from build123d import *

# Parameters (mm, degrees)
SKETCH1_W           = 800
SKETCH1_H           = 1200
BOSS_EXTRUDE1_DEPTH = 100
SKETCH2_W           = 40
SKETCH2_H           = 40
CUT_EXTRUDE1_DEPTH  = 1269.857754045
LPATTERN1_COUNT     = 5
LPATTERN1_PITCH     = 90
LPATTERN1_COL_COUNT = 5
LPATTERN1_COL_PITCH = 90


with BuildPart() as part:
    # Sketch1 → Boss-Extrude1 (new body)
    with BuildSketch(Plane.XY):
        Rectangle(SKETCH1_W, SKETCH1_H)
    extrude(amount=BOSS_EXTRUDE1_DEPTH)

    # Sketch2 → Cut-Extrude1 (cut, through all)
    with BuildSketch(Plane.XZ.offset(600)):
        with Locations((0, 100)):
            Rectangle(SKETCH2_W, SKETCH2_H)
    cut_extrude1 = extrude(amount=-CUT_EXTRUDE1_DEPTH, mode=Mode.SUBTRACT)

    # LPattern1: Cut-Extrude1 ×5
    with Locations(*[(i * LPATTERN1_PITCH, 0, 0) for i in range(1, LPATTERN1_COUNT)]):
        add(cut_extrude1, mode=Mode.SUBTRACT)

    # LPattern1 col: Cut-Extrude1 ×5
    with Locations(*[(-i * LPATTERN1_COL_PITCH, 0, 0) for i in range(1, LPATTERN1_COL_COUNT)]):
        add(cut_extrude1, mode=Mode.SUBTRACT)


solid = part.part
Verification items for the finished model (mm, model axes). A direction names the side the tool comes from. Coordinates: 2 decimals unless noted, no trailing zeros. Put each result on its own line as item: value. Start each with the question number.
1. Go/stop test with a flat-tipped pin: pin 1 Ø2 at (x, y) = (-285.5, -417.5) entering from +Z. Record where the tip stops, or that it passes through.
2. Material ranges on L1, parallel to Z at x = 287, y = 496, recorded low to high. Write a range as [from, to].
3. Access from +Z, -Z, +X, -X, +Y, -Y to the whole of each face (thin tool, end or side, straight path). Record for faces 1 (the flat face through (135, 8, 100)), 2 (the flat face through (-90, -8, 80)).
4. Mould release check, pull along X, two halves, no side actions. Record for faces 3 (the flat face through (-45, 8, 100)), 4 (the flat face through (-400, -8, 49)), 5 (the flat face through (-360, -8, 80)), 6 (the flat face through (270, -8, 80)): released by +X, released by -X, zero draft, split by the parting line, or undercut.
Computed:
1. pin 1: z = 80
2. L1: [0, 80]
3. face 1: +Z, +X, -X, +Y, -Y
3. face 2: +Z, +Y, -Y
4. face 3: zero draft
4. face 4: released by -X
4. face 5: undercut
4. face 6: undercut
